```python
from build123d import *

# Parameters (mm, degrees)
L_BRACKET_BODY_DEPTH         = 17.5
UPRIGHT_SLOT_DEPTH           = 35
CORNER_SUPPORT_BOSS_SKETCH_R = 8
CORNER_SUPPORT_BOSS_DEPTH    = 8
DOWEL_HOLE_10_D              = 10


with BuildPart() as part:
    # L-Bracket Profile Sketch → L-Bracket Body (new, symmetric)
    with BuildSketch(Plane(origin=(0, 0, 0), x_dir=(0, 0, -1), z_dir=(1, 0, 0))):
        Polygon((0, 0), (30, 0), (30, 10), (7, 10), (7, 55), (13, 55), (13, 75), (0, 75), align=None)
    extrude(amount=L_BRACKET_BODY_DEPTH, both=True)

    # Upright Slot Sketch → Upright Slot (cut)
    with BuildSketch(Plane(origin=(0, 0, -13), x_dir=(-1, 0, 0), z_dir=(0, 0, -1))):
        with BuildLine():
            Line((-5.5, 70), (5.5, 70))
            ThreePointArc((5.5, 70), (10.5, 65), (5.5, 60))
            Line((5.5, 60), (-5.5, 60))
            ThreePointArc((-5.5, 60), (-10.5, 65), (-5.5, 70))
        make_face()
    extrude(amount=-UPRIGHT_SLOT_DEPTH, mode=Mode.SUBTRACT)

    # Corner Support Boss Sketch → Corner Support Boss (add)
    with BuildSketch(Plane(origin=(0, 0, -7), x_dir=(-1, 0, 0), z_dir=(0, 0, -1))):
        with BuildLine():
            Line((-3, 16.837553419), (-3, 10))
            Line((-3, 10), (3, 10))
            Line((3, 10), (3, 16.837553419))
            ThreePointArc((3, 16.837553419), (0, 43.5), (-3, 16.837553419))
        make_face()
        with Locations((0, 30)):
            Circle(CORNER_SUPPORT_BOSS_SKETCH_R, mode=Mode.SUBTRACT)
    extrude(amount=CORNER_SUPPORT_BOSS_DEPTH)

    # Dowel Hole Ø10 (through all)
    with Locations(Plane(origin=(0, 10, 0), x_dir=(1, 0, 0), z_dir=(0, 1, 0))):
        with Locations((-10.5, 22.240638775), (10.5, 22.240638775)):
            Hole(DOWEL_HOLE_10_D / 2)


solid = part.part
```
Here's how the part is built. I have some questions about the finished solid (model axes, mm). A direction names the side the tool comes from. Give positions to 0.01 mm unless a question says otherwise; leave off trailing zeros. Order: outer loops, then holes, each group sorted by start corner. A loop starts at its lowest first (then second) coordinate and runs counter-clockwise, first axis right, second up. Notation, with made-up numbers: (31, 73.25) - (63, 73.25) arc R31 cw to (63, 101.25) - close; hole circle Ø7 at (-7, 8). An arc over 180 degrees is marked (long way). Answer as a JSON object with one key per item and string values. Group by question number.
Item 1: If we section it at C-C on z = -19.25: Please give me the cut outline in (x, y).
Item 2: For P1, Ø8, axis at x = 4.5, y = 24, coming from the -Z side; P2, Ø6, axis at x = 4.5, y = 64, coming from the -Z side; P3, Ø7, axis at x = 8, z = -17, coming from the +Y side; P4, Ø3.5, axis at y = 12.5, z = -9.5, coming from the -X side, each with a flat end and sliding along its axis, tell me the tip position at first contact or that it passes through.
Item 3: If we section it at D-D on y = 30: Please give me the cut outline in (x, z).
Item 4: Please list where these lines run through material, in increasing order: probe 1 along Y at (x, z) = (0, -11); probe 2 along Z at (x, y) = (-10.5, 6.5); probe 3 along Y at (x, z) = (-2.5, -9.5).
Item 5: If we section it at B-B on x = 0: Please give me the cut outline in (y, z), and give its area (3 significant figures).
Item 6: Which directions (+Z, -Z, +X, -X, +Y, -Y) give clear straight access to the entire face, cutting with the end or side of a thin tool? Please do faces 1 (the flat face through (0, 70, -7)), 2 (the flat face through (-3, 13, -11)), 3 (the cylindrical face through (-0.55, 43.49, -10.94)), 4 (the flat face through (0, 58, -13)).
Item 7: If we section it at A-A on y = 65: Please give me the cut outline in (x, z), and give its area (3 significant figures).
Item 8: If we mould it in two halves opening along Y, with no side actions, what happens to faces 5 (the cylindrical face through (5.73, 4.93, -23.74)), 6 (the flat face through (3, 13, -11)), 7 (the cylindrical face through (10.5, 64.9, -6.6)), 8 (the flat face through (0, 0, -15))? For each: pulls with the +Y half, pulls with the -Y half, needs draft (parallel to the pull), parting line crosses it, or undercut.
Result set:
{
 "1": {"outline": "(-17.5, 0) - (-14.51, 0) - (-14.51, 10) - (-17.5, 10) - close; (-6.49, 0) - (6.49, 0) - (6.49, 10) - (-6.49, 10) - close; (14.51, 0) - (17.5, 0) - (17.5, 10) - (14.51, 10) - close"},
 "2": {"P1": "z = -15", "P2": "through", "P3": "y = 42.49", "P4": "x = -3"},
 "3": {"outline": "(-17.5, -7) - (-13.5, -7) - (-13.5, -15) - (-8, -15) - (-8, -7) - (8, -7) - (8, -15) - (13.5, -15) - (13.5, -7) - (17.5, -7) - (17.5, 0) - (-17.5, 0) - close"},
 "4": {"probe 1": "0 to 22, 38 to 43.5, 55 to 60, 70 to 75", "probe 2": "-30 to -27.24, -17.24 to 0", "probe 3": "0 to 22.4, 37.6 to 43.27, 55 to 60, 70 to 75"},
 "5": {"outline": "(0, -30) - (10, -30) - (10, -15) - (22, -15) - (22, -7) - (38, -7) - (38, -15) - (43.5, -15) - (43.5, -7) - (55, -7) - (55, -13) - (60, -13) - (60, 0) - (0, 0) - close; (70, -13) - (75, -13) - (75, 0) - (70, 0) - close", "area": "885 mm²"},
 "6": {"face 1": "+Z, -Z", "face 2": "-Z, -X", "face 3": "-Z", "face 4": "-Z, +X, -X, +Y"},
 "7": {"outline": "(-17.5, -13) - (-10.5, -13) - (-10.5, 0) - (-17.5, 0) - close; (10.5, -13) - (17.5, -13) - (17.5, 0) - (10.5, 0) - close", "area": "182 mm²"},
 "8": {"face 5": "needs draft", "face 6": "undercut", "face 7": "undercut", "face 8": "pulls with the -Y half"}
}
